```python
from build123d import *

# Parameters (mm, degrees)
BOSS_EXTRUDE1_DEPTH        = 1
F_4_2_4_2_DIAMETER_HOLE1_D = 4.2


with BuildPart() as part:
    # Sketch1 → Boss-Extrude1 (new, symmetric)
    with BuildSketch(Plane.XY):
        with BuildLine():
            Line((0, 6), (84, 6))
            ThreePointArc((84, 6), (90, 0), (84, -6))
            Line((84, -6), (0, -6))
            ThreePointArc((0, -6), (-6, 0), (0, 6))
        make_face()
    extrude(amount=BOSS_EXTRUDE1_DEPTH, both=True)

    # Ø4.2 (4.2) Diameter Hole1 (through all)
    with Locations(Plane.XY.offset(1)):
        with Locations((0, 0), (84, 0)):
            Hole(F_4_2_4_2_DIAMETER_HOLE1_D / 2)


solid = part.part
```
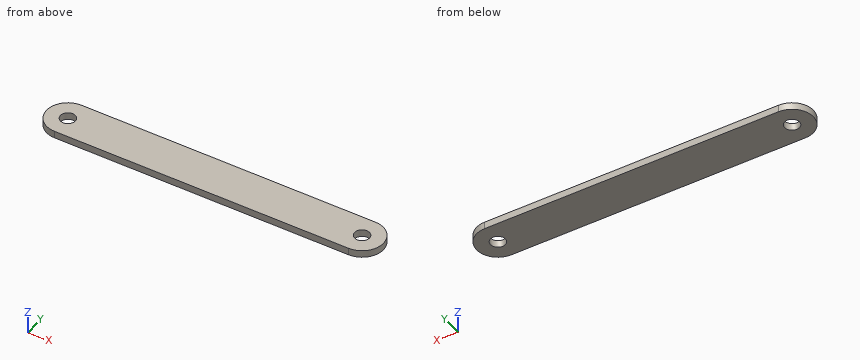
Verification items for the finished model (mm, model axes). Round coordinates to 2 decimals unless told otherwise and drop trailing zeros. Write each loop counter-clockwise with the first axis right and the second up, starting at its lowest first coordinate (ties: lowest second). Pieces come first, ordered by that corner, then holes.
1. Section check C-C on y = -4.5. Enter the section's corners in (x, z).
2. Scan lines: L1, parallel to X at y = -0.25, z = -0.6; L2, parallel to Y at x = 0, z = -0.05; L3, parallel to X at y = 0.5, z = -0.5. Record each from-to range of solid material in increasing order.
3. Gauge pin test, flat end, axial feed: P1, Ø1, axis at y = 4, z = -0.5, coming from the -X side. Record the tip position at first contact, or that the pin passes through.
4. Section check B-B on z = 0.05. Enter the section's corners in (x, y), plus the area to 3 significant figures.
5. Section check A-A on y = 0. Enter the section's corners in (x, z).
Answer:
1. outline: (-3.97, -1) - (87.97, -1) - (87.97, 1) - (-3.97, 1) - close
2. L1: x = -5.99 to -2.09, 2.09 to 81.91, 86.09 to 89.99
2. L2: y = -6 to -2.1, 2.1 to 6
2. L3: x = -5.98 to -2.04, 2.04 to 81.96, 86.04 to 89.98
3. P1: stops at x = -4.87
4. outline: (0, -6) - (84, -6) arc R6 ccw to (84, 6) - (0, 6) arc R6 ccw to start; hole circle Ø4.2 at (0, 0); hole circle Ø4.2 at (84, 0)
4. area: 1,090 mm2
5. outline: (-6, -1) - (-2.1, -1) - (-2.1, 1) - (-6, 1) - close; (2.1, -1) - (81.9, -1) - (81.9, 1) - (2.1, 1) - close; (86.1, -1) - (90, -1) - (90, 1) - (86.1, 1) - close
